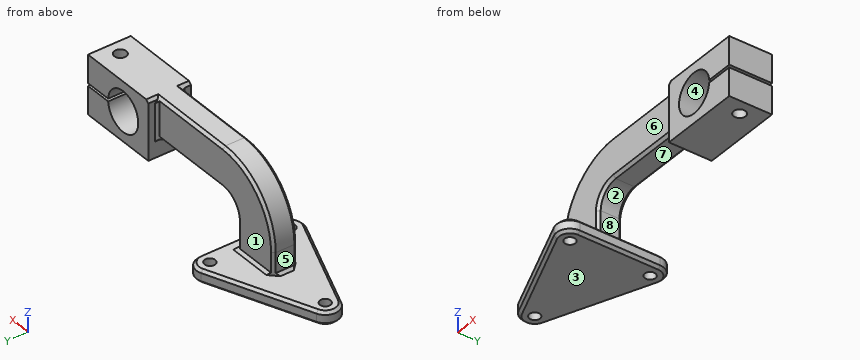
```python
from build123d import *

# Parameters (mm, degrees)
CLAMP_BLOCK_SKETCH_W       = 60
CLAMP_BLOCK_SKETCH_H       = 32
CLAMP_BLOCK_DEPTH          = 44
SPLIT_BORE_CUT_DEPTH       = 44
CLAMP_BOLT_HOLE_SKETCH_R   = 4.5
CLAMP_BOLT_HOLE_DEPTH      = 60
ARM_SKETCH_W               = 30
ARM_SKETCH_H               = 18
ARM_DEPTH                  = 65
ARM_BEND_DEPTH             = 18
MOUNTING_FLANGE_DEPTH      = 10
FLANGE_HOLES_SKETCH_R      = 4
FLANGE_HOLES_3X_8_DEPTH    = 10
ARM_BEND_CHAMFER_SIZE      = 2
CLAMP_BLOCK_CHAMFER_A_SIZE = 2
ARM_CLAMP_CHAMFER_A_SIZE   = 2
ARM_EDGE_CHAMFER_SIZE      = 2
ARM_CLAMP_CHAMFER_B_SIZE   = 2
CLAMP_BLOCK_CHAMFER_B_SIZE = 2
ARM_FLANGE_CHAMFER_A_SIZE  = 2
BEND_FLANGE_CHAMFER_A_SIZE = 2
ARM_FLANGE_CHAMFER_B_SIZE  = 2
BEND_FLANGE_CHAMFER_B_SIZE = 2
FLANGE_EDGE_CHAMFER_SIZE   = 2
BEND_EDGE_CHAMFER_A_SIZE   = 2
BEND_EDGE_CHAMFER_B_SIZE   = 2
ARM_CLAMP_CHAMFER_C_SIZE   = 2


with BuildPart() as part:
    # Clamp Block Sketch → Clamp Block (new body)
    with BuildSketch(Plane.XY):
        with Locations((30, -16)):
            Rectangle(CLAMP_BLOCK_SKETCH_W, CLAMP_BLOCK_SKETCH_H)
    extrude(amount=-CLAMP_BLOCK_DEPTH)

    # Split Bore Sketch → Split Bore Cut (cut)
    with BuildSketch(Plane.XZ.offset(32)):
        with BuildLine():
            Line((60, -21), (60, -23))
            Line((60, -23), (39.966629547, -23))
            ThreePointArc((39.966629547, -23), (10, -22), (39.966629547, -21))
            Line((39.966629547, -21), (60, -21))
        make_face()
    extrude(amount=-SPLIT_BORE_CUT_DEPTH, mode=Mode.SUBTRACT)

    # Clamp Bolt Hole Sketch → Clamp Bolt Hole (cut)
    with BuildSketch(Plane.XY):
        with Locations(Location((49.119785918, -16, 0), (0, 0, 180))):
            Circle(CLAMP_BOLT_HOLE_SKETCH_R)
    extrude(amount=-CLAMP_BOLT_HOLE_DEPTH, mode=Mode.SUBTRACT)

    # Arm Sketch → Arm (add)
    with BuildSketch(Plane.ZY):
        with Locations((-15, -16)):
            Rectangle(ARM_SKETCH_W, ARM_SKETCH_H)
    extrude(amount=ARM_DEPTH)

    # Arm Bend Sketch → Arm Bend (add)
    with BuildSketch(Plane.XZ.offset(25)):
        with BuildLine():
            Line((-115, -67), (-80, -67))
            Line((-80, -67), (-80, -45))
            ThreePointArc((-80, -45), (-75.606601718, -34.393398282), (-65, -30))
            Line((-65, -30), (-65, 0))
            ThreePointArc((-65, 0), (-100.355339059, -14.644660941), (-115, -50))
            Line((-115, -50), (-115, -67))
        make_face()
    extrude(amount=-ARM_BEND_DEPTH)

    # Mounting Flange Sketch → Mounting Flange (add)
    with BuildSketch(Plane(origin=(0, 0, -67), x_dir=(-1, 0, 0), z_dir=(0, 0, -1))):
        with BuildLine():
            Line((83.713906764, 23.284766909), (158.713906764, -6.715233091))
            ThreePointArc((158.713906764, -6.715233091), (165, -16), (158.713906764, -25.284766909))
            Line((158.713906764, -25.284766909), (83.713906764, -55.284766909))
            ThreePointArc((83.713906764, -55.284766909), (74.393711907, -54.280672305), (70, -46))
            Line((70, -46), (70, 14))
            ThreePointArc((70, 14), (74.393711907, 22.280672305), (83.713906764, 23.284766909))
        make_face()
    extrude(amount=MOUNTING_FLANGE_DEPTH)

    # Flange Holes Sketch → Flange Holes 3xØ8 (cut)
    with BuildSketch(Plane(origin=(0, 0, -77), x_dir=(-1, 0, 0), z_dir=(0, 0, -1))):
        with Locations((80, 14)):
            Circle(FLANGE_HOLES_SKETCH_R)
        with Locations((155, -16)):
            Circle(FLANGE_HOLES_SKETCH_R)
        with Locations((80, -46)):
            Circle(FLANGE_HOLES_SKETCH_R)
    extrude(amount=-FLANGE_HOLES_3X_8_DEPTH, mode=Mode.SUBTRACT)

    # Arm-Bend Chamfer
    arm_bend_chamfer_edges = [part.edges().sort_by_distance(p)[0] for p in [
        (-32.5, -25, 0),
        (-100.355339059, -25, -14.644660941),
        (-115, -25, -58.5),
    ]]
    chamfer(arm_bend_chamfer_edges, length=ARM_BEND_CHAMFER_SIZE)

    # Clamp Block Chamfer A
    clamp_block_chamfer_a_edges = [part.edges().sort_by_distance(p)[0] for p in [
        (0, -27.5, 0),
    ]]
    chamfer(clamp_block_chamfer_a_edges, length=CLAMP_BLOCK_CHAMFER_A_SIZE)

    # Arm-Clamp Chamfer A
    arm_clamp_chamfer_a_edges = [part.edges().sort_by_distance(p)[0] for p in [
        (0, -25, -16),
    ]]
    chamfer(arm_clamp_chamfer_a_edges, length=ARM_CLAMP_CHAMFER_A_SIZE)

    # Arm Edge Chamfer
    arm_edge_chamfer_edges = [part.edges().sort_by_distance(p)[0] for p in [
        (-32.5, -7, 0),
        (-115, -7, -58.5),
        (-100.355339059, -7, -14.644660941),
    ]]
    chamfer(arm_edge_chamfer_edges, length=ARM_EDGE_CHAMFER_SIZE)

    # Arm-Clamp Chamfer B
    arm_clamp_chamfer_b_edges = [part.edges().sort_by_distance(p)[0] for p in [
        (0, -7, -16),
    ]]
    chamfer(arm_clamp_chamfer_b_edges, length=ARM_CLAMP_CHAMFER_B_SIZE)

    # Clamp Block Chamfer B
    clamp_block_chamfer_b_edges = [part.edges().sort_by_distance(p)[0] for p in [
        (0, -4.5, 0),
    ]]
    chamfer(clamp_block_chamfer_b_edges, length=CLAMP_BLOCK_CHAMFER_B_SIZE)

    # Arm-Flange Chamfer A
    arm_flange_chamfer_a_edges = [part.edges().sort_by_distance(p)[0] for p in [
        (-96.5, -25, -67),
        (-74.393711907, 22.280672305, -67),
        (-70, -16, -67),
        (-74.393711907, -54.280672305, -67),
        (-121.213906764, -40.284766909, -67),
        (-165, -16, -67),
        (-121.213906764, 8.284766909, -67),
    ]]
    chamfer(arm_flange_chamfer_a_edges, length=ARM_FLANGE_CHAMFER_A_SIZE)

    # Bend-Flange Chamfer A
    bend_flange_chamfer_a_edges = [part.edges().sort_by_distance(p)[0] for p in [
        (-115, -16, -67),
    ]]
    chamfer(bend_flange_chamfer_a_edges, length=BEND_FLANGE_CHAMFER_A_SIZE)

    # Arm-Flange Chamfer B
    arm_flange_chamfer_b_edges = [part.edges().sort_by_distance(p)[0] for p in [
        (-96.5, -7, -67),
    ]]
    chamfer(arm_flange_chamfer_b_edges, length=ARM_FLANGE_CHAMFER_B_SIZE)

    # Bend-Flange Chamfer B
    bend_flange_chamfer_b_edges = [part.edges().sort_by_distance(p)[0] for p in [
        (-80, -16, -67),
    ]]
    chamfer(bend_flange_chamfer_b_edges, length=BEND_FLANGE_CHAMFER_B_SIZE)

    # Flange Edge Chamfer
    flange_edge_chamfer_edges = [part.edges().sort_by_distance(p)[0] for p in [
        (-74.393711907, 22.280672305, -77),
        (-70, -16, -77),
        (-74.393711907, -54.280672305, -77),
        (-121.213906764, -40.284766909, -77),
        (-165, -16, -77),
        (-121.213906764, 8.284766909, -77),
    ]]
    chamfer(flange_edge_chamfer_edges, length=FLANGE_EDGE_CHAMFER_SIZE)

    # Bend Edge Chamfer A
    bend_edge_chamfer_a_edges = [part.edges().sort_by_distance(p)[0] for p in [
        (-80, -25, -55),
        (-33.5, -25, -30),
        (-75.606601718, -25, -34.393398282),
    ]]
    chamfer(bend_edge_chamfer_a_edges, length=BEND_EDGE_CHAMFER_A_SIZE)

    # Bend Edge Chamfer B
    bend_edge_chamfer_b_edges = [part.edges().sort_by_distance(p)[0] for p in [
        (-80, -7, -55),
        (-33.5, -7, -30),
        (-75.606601718, -7, -34.393398282),
    ]]
    chamfer(bend_edge_chamfer_b_edges, length=BEND_EDGE_CHAMFER_B_SIZE)

    # Arm-Clamp Chamfer C
    arm_clamp_chamfer_c_edges = [part.edges().sort_by_distance(p)[0] for p in [
        (0, -16, -30),
    ]]
    chamfer(arm_clamp_chamfer_c_edges, length=ARM_CLAMP_CHAMFER_C_SIZE)


solid = part.part
```
Model file for the job. Use its own axes, mm. Face numbers are marked on the shaded views. A direction names the side the tool comes from. Round coordinates to 2 decimals unless told otherwise and drop trailing zeros. Order: outer loops, then holes, each group sorted by start corner. A loop starts at its lowest first (then second) coordinate and runs counter-clockwise, first axis right, second up. Notation, with made-up numbers: (53, 3) -> (105, 3) arc R17 ccw to (105, 19) -> close; hole circle Ø11 at (37, 39.5). An arc over 180 degrees is marked (long way). Use one line per item in the form item = value.
Item 1: Cut at B-B, the plane x = -53. Write the cut outline in (y, z).
Returned:
outline = (-25, -28) -> (-23, -30) -> (-9, -30) -> (-7, -28) -> (-7, -2) -> (-9, 0) -> (-23, 0) -> (-25, -2) -> close
Item 2: Flat gauge pins, fed straight in: pin 1 Ø8 at (y, z) = (2.5, -42) entering from -X; pin 2 Ø9.5 at (y, z) = (-10.5, -24) entering from -X; pin 3 Ø10.5 at (x, y) = (-80, 14) entering from +Z; pin 4 Ø7 at (x, y) = (49.12, -16) entering from +Z. Where does each tip first touch, or does it go through?
Returned:
pin_1 = 0
pin_2 = -110.26
pin_3 = -67
pin_4 = through
Item 3: Cut at D-D, the plane x = -135.5. Write the cut outline in (y, z).
Returned:
outline = (-34.57, -75) -> (-32.42, -77) -> (0.42, -77) -> (2.57, -75) -> (2.57, -69) -> (0.42, -67) -> (-32.42, -67) -> (-34.57, -69) -> close
Item 4: Pull direction Z, two halves, no side cores. Call the marked faces 1, 2, 3 and 4: released by +Z, released by -Z, zero draft, split by the parting line, or undercut.
Returned:
face_1 = zero draft
face_2 = undercut
face_3 = released by -Z
face_4 = undercut
Item 5: Tool access for the marked faces 5, 6, 7 and 8: list every direction of +Z, -Z, +X, -X, +Y, -Y with a clear straight run to the whole face (end or side of a thin tool).
Returned:
face_5 = +Z, -X, +Y, -Y
face_6 = +Z, -X, -Y
face_7 = -Z, +Y, -Y
face_8 = +X, +Y, -Y
Item 6: Cut at A-A, the plane x = 23. Write the cut outline in (y, z).
Returned:
outline = (-32, -44) -> (0, -44) -> (0, -36.87) -> (-32, -36.87) -> close; (-32, -7.13) -> (0, -7.13) -> (0, 0) -> (-32, 0) -> close
Item 7: Cut at C-C, the plane y = -16. Give the number of separate pieces and of enclosed holes in the cut face, and give its area (3 significant figures).
Returned:
separate_pieces = 4
enclosed_holes = 0
area = 6,640 mm^2
Item 8: Drill centre lines: line 1 (Y direction, x = -154.5, z = -71.5); line 2 (Y direction, x = -39, z = -23.5); line 3 (Y direction, x = 4, z = -37). Where is each one in solid material? Low to high.
Returned:
line_1 = -26.97 to -19.97, -12.03 to -5.03
line_2 = -25 to -7
line_3 = -32 to 0
